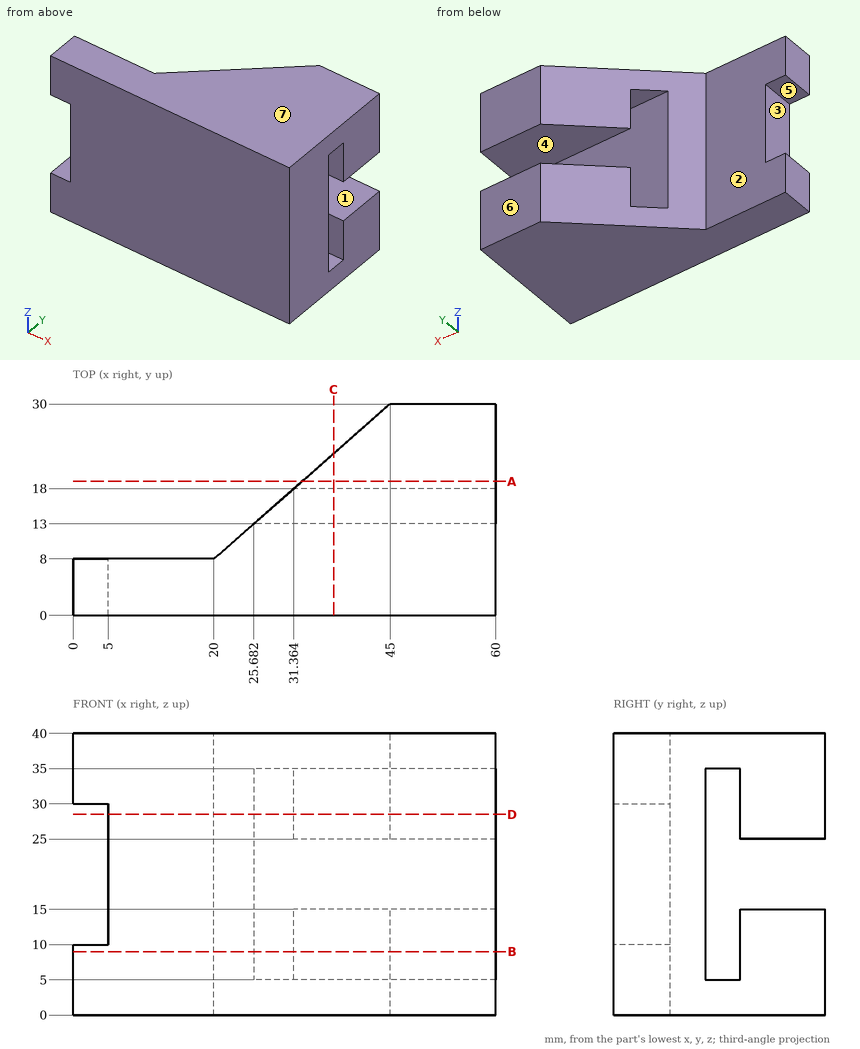
Study the drawing (mm; zero at the part's minimum x, y, z) and answer. A direction names the side the tool comes from. Coordinates: 2 decimals unless noted, no trailing zeros. Loops run counter-clockwise (first coordinate to the right, second up) from the corner with the lowest first, then second, coordinate; pieces in that order, holes last. Notation, with made-up numbers: (-27, 72) -> (24, 72) arc R21 ccw to (24, 82) -> close; hole circle Ø11 at (70, 53.5). An arc over 180 degrees is marked (long way). Write item = value, one per line. Start each with the question number.
1) The part is cut by section A-A, the plane y = 19. Determine the outline of the cut face in (x, z).
2) For the marked faces 1, 2 and 3, determine the directions among +Z, -Z, +X, -X, +Y, -Y from which every point of the face is accessible in a straight line to the end or side of a thin tool.
3) The part is cut by section D-D, the plane z = 28.5. Determine the outline of the cut face in (x, y).
4) The part is cut by section C-C, the plane x = 37. Determine the outline of the cut face in (y, z), plus the area to 3 significant figures.
5) Find the intervals of material crossed by L1, parallel to Z at x = 50, y = 19; L2, parallel to Y at x = 56.5, z = 28.5; L3, parallel to Z at x = 40, y = 13.75, in increasing order. Write a range as from..to.
6) The mould has two halves that part along Z. Classify the marked faces 4, 5, 6 and 7: pulls with the +Z half, pulls with the -Z half, needs draft (parallel to the pull), parting line crosses it, or undercut.
7) Given P1, Ø5, axis at x = 28.5, z = 18.5, coming from the +Y side; P2, Ø6, axis at x = 5.5, z = 13, coming from the +Y side; P3, Ø9, axis at y = 4.5, z = 15.5, coming from the -X side, each flat-ended and moving along its own axis, determine where each tip first touches the part or whether it passes through.
8) The part is cut by section B-B, the plane z = 9. Determine the outline of the cut face in (x, y).
Result:
q1.outline = (32.5, 0) -> (60, 0) -> (60, 15) -> (32.5, 15) -> close; (32.5, 25) -> (60, 25) -> (60, 40) -> (32.5, 40) -> close
q2.face_1 = +X, -X, +Y
q2.face_2 = +Z, -Z, -X, +Y
q2.face_3 = -X, +Y, -Y
q3.outline = (5, 0) -> (60, 0) -> (60, 13) -> (25.68, 13) -> (20, 8) -> (5, 8) -> close; (31.36, 18) -> (60, 18) -> (60, 30) -> (45, 30) -> close
q4.outline = (0, 0) -> (22.96, 0) -> (22.96, 15) -> (18, 15) -> (18, 5) -> (13, 5) -> (13, 35) -> (18, 35) -> (18, 25) -> (22.96, 25) -> (22.96, 40) -> (0, 40) -> close
q4.area = 719 mm²
q5.L1 = 0..15, 25..40
q5.L2 = 0..13, 18..30
q5.L3 = 0..5, 35..40
q6.face_4 = undercut
q6.face_5 = undercut
q6.face_6 = needs draft
q6.face_7 = pulls with the +Z half
q7.P1 = 13
q7.P2 = 8
q7.P3 = 5
q8.outline = (0, 0) -> (60, 0) -> (60, 13) -> (25.68, 13) -> (20, 8) -> (0, 8) -> close; (31.36, 18) -> (60, 18) -> (60, 30) -> (45, 30) -> close
